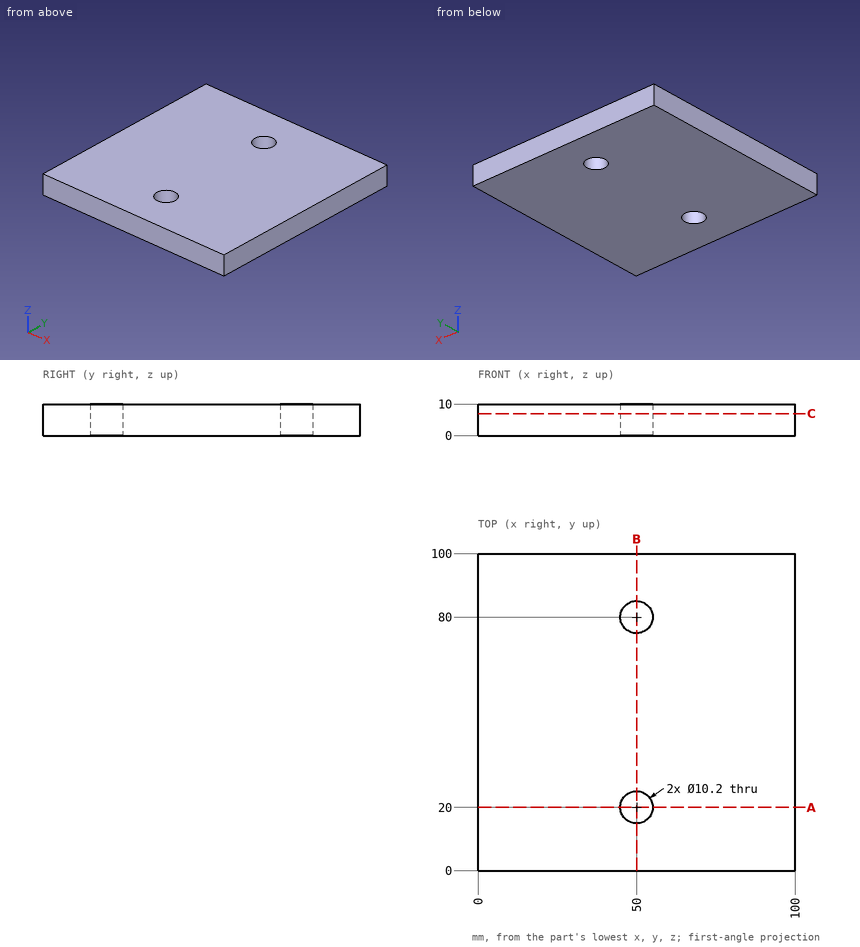
Print and shaded views of the part. All mm, measured from the part's lowest x, y and z. Coordinates: 2 decimals unless noted, no trailing zeros. Loops run counter-clockwise (first coordinate to the right, second up) from the corner with the lowest first, then second, coordinate; pieces in that order, holes last. Notation, with made-up numbers: (-8, 77.5) - (19, 77.5) arc R29 ccw to (19, 116.5) - close; hole circle Ø2 at (-16.5, 18). An arc over 180 degrees is marked (long way). Write item = value, one per line. Start each with the question number.
Item 1: Saw through at B-B, the plane x = 50. List the corners of the cut face in (y, z).
Item 2: Saw through at C-C, the plane z = 7. List the corners of the cut face in (x, y).
Item 3: Saw through at A-A, the plane y = 20. List the corners of the cut face in (x, z).
Item 4: Wall check: probe 1 along Y at (x, z) = (50, 6.75); probe 2 along Y at (x, z) = (51.5, 9.5); probe 3 along X at (y, z) = (79, 2.25). Give the ranges that are in metal, low to high. Write a range as [from, to].
Item 5: Drop flat-ended pins along their axis: pin 1 Ø8 at (x, y) = (69, 71) entering from -Z; pin 2 Ø8 at (x, y) = (50, 80) entering from +Z. Give the stop position or say it passes through.
Answers:
q1.outline = (0, 0) - (14.9, 0) - (14.9, 10) - (0, 10) - close; (25.1, 0) - (74.9, 0) - (74.9, 10) - (25.1, 10) - close; (85.1, 0) - (100, 0) - (100, 10) - (85.1, 10) - close
q2.outline = (0, 0) - (100, 0) - (100, 100) - (0, 100) - close; hole circle Ø10.2 at (50, 20); hole circle Ø10.2 at (50, 80)
q3.outline = (0, 0) - (44.9, 0) - (44.9, 10) - (0, 10) - close; (55.1, 0) - (100, 0) - (100, 10) - (55.1, 10) - close
q4.probe_1 = [0, 14.9], [25.1, 74.9], [85.1, 100]
q4.probe_2 = [0, 15.13], [24.87, 75.13], [84.87, 100]
q4.probe_3 = [0, 45], [55, 100]
q5.pin_1 = 0
q5.pin_2 = through
